The model under review builds one solid part; all positions refer to its coordinate system, in mm. Face numbers are marked on the shaded views. A direction names the side the tool comes from. Give positions to 0.01 mm unless a question says otherwise; leave off trailing zeros. Loops run counter-clockwise (first coordinate to the right, second up) from the corner with the lowest first, then second, coordinate; pieces in that order, holes last. Notation, with made-up numbers: M 1,6.5 L 54,6.5 A24 ccw 54,38.5 Z; hole C -1.75,-4 d10. An arc over 180 degrees is marked long. Put each result on its own line as item: value. Start each with the question number.
```python
from build123d import *

# Parameters (mm, degrees)
BOSS_EXTRUDE1_DEPTH = 31.5
SKETCH2_W           = 30
SKETCH2_H           = 3
BOSS_EXTRUDE2_DEPTH = 63
SKETCH3_R           = 1.75
CUT_EXTRUDE1_DEPTH  = 50
FILLET1_R           = 4


with BuildPart() as part:
    # Sketch1 → Boss-Extrude1 (new, symmetric)
    with BuildSketch(Plane.XY):
        Polygon((0, 0), (-6.189633375, 18), (-47.911924672, 41.911648908), (-1.016937138, 29.024958443), (12.517623262, 0), align=None)
    extrude(amount=BOSS_EXTRUDE1_DEPTH, both=True)

    # Sketch2 → Boss-Extrude2 (add)
    with BuildSketch(Plane.XY.offset(31.5)):
        with Locations((15, 1.5)):
            Rectangle(SKETCH2_W, SKETCH2_H)
    extrude(amount=-BOSS_EXTRUDE2_DEPTH)

    # Sketch3 → Cut-Extrude1 (cut)
    with BuildSketch(Plane(origin=(0, 3, 0), x_dir=(1, 0, 0), z_dir=(0, 1, 0))):
        with Locations(Location((20.559350144, 18.5, 0), (0, 0, 270))):
            Circle(SKETCH3_R)
        with Locations(Location((20.559350144, 0.5, 0), (0, 0, 270))):
            Circle(SKETCH3_R)
        with Locations(Location((20.559350144, -17.5, 0), (0, 0, 270))):
            Circle(SKETCH3_R)
    extrude(amount=-CUT_EXTRUDE1_DEPTH, mode=Mode.SUBTRACT)

    # Fillet1
    fillet1_edges = [part.edges().sort_by_distance(p)[0] for p in [
        (30, 1.5, 31.5),
        (30, 1.5, -31.5),
    ]]
    fillet(fillet1_edges, radius=FILLET1_R)


solid = part.part
```
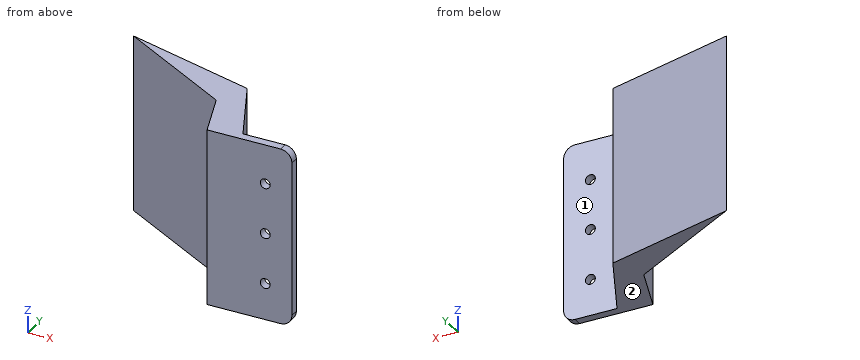
Item 1: Consider section D-D, the plane y = 9. Write out the cut boundary in (x, z).
Item 2: Consider section A-A, the plane z = 17.5. Write out the cut boundary in (x, y), plus the area to 3 significant figures.
Item 3: Consider section B-B, the plane z = 26.5. Write out the cut boundary in (x, y), plus the area to 3 significant figures.
Item 4: To check wall thickness, follow L1, parallel to X at y = 1, z = 0; L2, parallel to Y at x = 22.5, z = 26; L3, parallel to X at y = 2.4, z = -0.5. State the ranges of each line that lie inside material, in increasing order. Write a range as [from, to].
Item 5: Clearance check with flat-ended pins moving along their axes: pin 1 Ø10 at (x, z) = (17, 3) entering from +Y; pin 2 Ø3 at (y, z) = (17.5, 7) entering from -X; pin 3 Ø4 at (y, z) = (8, 4) entering from -X. State where each tip first meets the part, or that it passes through.
Item 6: Tool access review of the marked faces 1 and 2: name each direction out of +Z, -Z, +X, -X, +Y, -Y from which nothing blocks a thin tool from reaching the whole face with its end or side.
Item 7: Consider section C-C, the plane x = 17.5. Write out the cut boundary in (y, z), plus the area to 3 significant figures.
Report:
1. outline: M -3.09,-31.5 L 8.32,-31.5 L 8.32,31.5 L -3.09,31.5 Z
2. outline: M -47.91,41.91 L -6.19,18 L 0,0 L 18.81,0 L 18.81,3 L 11.12,3 L -1.02,29.02 Z; M 22.31,0 L 30,0 L 30,3 L 22.31,3 Z
2. area: 598 mm²
3. outline: M -47.91,41.91 L -6.19,18 L 0,0 L 30,0 L 30,3 L 11.12,3 L -1.02,29.02 Z
3. area: 609 mm²
4. L1: [-0.34, 18.88], [22.24, 30]
4. L2: [0, 3]
4. L3: [-0.83, 18.81], [22.31, 30]
5. pin 1: y = 3
5. pin 2: x = -7.93
5. pin 3: x = -3.44
6. face 1: +Z, -Z, +X, +Y
6. face 2: -Z, +X, -X, +Y, -Y
7. outline: M 0,-31.5 L 3,-31.5 L 3,31.5 L 0,31.5 Z
7. area: 189 mm²
